```python
from build123d import *

# Parameters (mm, degrees)
EXTRUDE_1_DEPTH     = 3
FILLET_1_R          = 3
SKETCH_2_W          = 12
SKETCH_2_H          = 10
CUT_EXTRUDE_1_DEPTH = 57.903426962


with BuildPart() as part:
    # 草图1 → 凸台-拉伸1 (new body)
    with BuildSketch(Plane(origin=(0, 0, 0), x_dir=(0, 0, -1), z_dir=(1, 0, 0))):
        Polygon((-22, 50), (-27, 45), (-27, 0), (0, 0), (0, 50), align=None)
    extrude(amount=EXTRUDE_1_DEPTH)

    # 圆角1
    fillet_1_edges = [part.edges().sort_by_distance(p)[0] for p in [
        (1.5, 0, 0),
    ]]
    fillet(fillet_1_edges, radius=FILLET_1_R)

    # 草图2 → 切除-拉伸1 (cut, through all)
    with BuildSketch(Plane(origin=(3, 0, 0), x_dir=(0, 0, -1), z_dir=(1, 0, 0))):
        with Locations((-14, 35)):
            Rectangle(SKETCH_2_W, SKETCH_2_H)
    extrude(amount=-CUT_EXTRUDE_1_DEPTH, mode=Mode.SUBTRACT)


solid = part.part
```
The listing builds one solid part. Answer for the finished solid, in the listing's coordinates (mm). A direction names the side the tool comes from. Give positions to 0.01 mm unless a question says otherwise; leave off trailing zeros. Loops run counter-clockwise (first coordinate to the right, second up) from the corner with the lowest first, then second, coordinate; pieces in that order, holes last. Notation, with made-up numbers: (63, -28) - (74, -28) arc R24 ccw to (74, 1) - close; hole circle Ø3 at (9, -4.5). An arc over 180 degrees is marked (long way). Return JSON: item names as keys, results as strings. Group by question number.
1. Find section B-B (y = 31). Write down the section's boundary in (x, z).
2. Determine the mould class of faces 3 (the flat face through (0, 25, 14)), 4 (the flat face through (1, 50, 11)), 5 (the flat face through (2, 35, 8)) for opening direction Y: pulls with the +Y half, pulls with the -Y half, needs draft (parallel to the pull), parting line crosses it, or undercut.
3. Find section C-C (x = 1). Write down the section's boundary in (y, z).
4. Find section D-D (z = 23.25). Write down the section's boundary in (x, y).
5. Straight lines are drawn through the part: line 1 (Y direction, x = 1.5, z = 13); line 2 (Z direction, x = 1.6, y = 30.5); line 3 (Z direction, x = 1, y = 46.5). For each, find the intervals that lie inside material, in ascending order. Write a range as [from, to].
6. Find section A-A (z = 17.5). Write down the section's boundary in (x, y), then the cut area to 3 significant figures.
7. Which of the six approach directions +Z, -Z, +X, -X, +Y, -Y give full straight-line access (tool end or side, diameter ignored) to faces 1 (the flat face through (2, 35, 20)), 2 (the cylindrical face through (1.52, 0.86, 0.9))?
Verdict:
{
 "1": {"outline": "(0, 0) - (3, 0) - (3, 8) - (0, 8) - close; (0, 20) - (3, 20) - (3, 27) - (0, 27) - close"},
 "2": {"face 3": "needs draft", "face 4": "pulls with the +Y half", "face 5": "undercut"},
 "3": {"outline": "(0, 3) arc R3 ccw to (3, 0) - (50, 0) - (50, 22) - (45, 27) - (0, 27) - close; hole (30, 8) - (40, 8) - (40, 20) - (30, 20) - close"},
 "4": {"outline": "(0, 0) - (3, 0) - (3, 48.75) - (0, 48.75) - close"},
 "5": {"line 1": "y = [0, 30], [40, 50]", "line 2": "z = [0, 8], [20, 27]", "line 3": "z = [0, 25.5]"},
 "6": {"outline": "(0, 0) - (3, 0) - (3, 30) - (0, 30) - close; (0, 40) - (3, 40) - (3, 50) - (0, 50) - close", "area": "120 mm^2"},
 "7": {"face 1": "+X, -X", "face 2": "-Z, +X, -X, -Y"}
}
